Input: dimensioned drawing with shaded views. Units: mm. Origin: part minimum x, y, z. Give positions to 0.01 mm unless a question says otherwise; leave off trailing zeros. Order: outer loops, then holes, each group sorted by start corner. A loop starts at its lowest first (then second) coordinate and runs counter-clockwise, first axis right, second up.
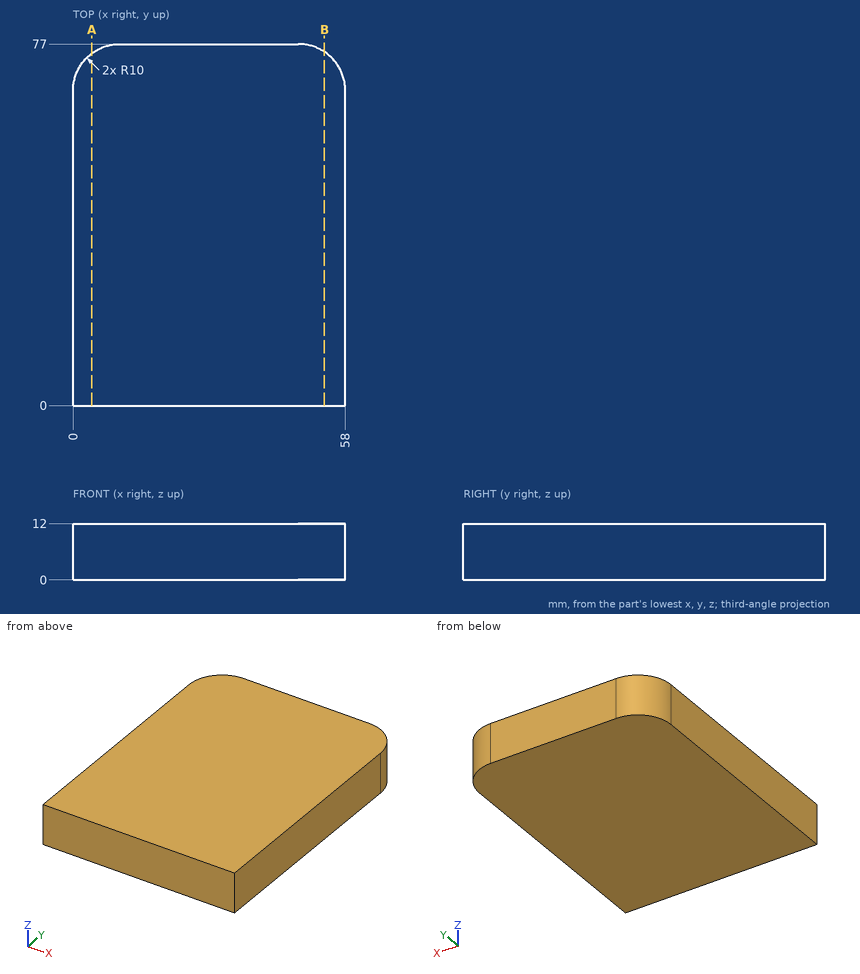
1) Line query: probe 1 along Y at (x, z) = (9.5, 0.75); probe 2 along Y at (x, z) = (49, 1.75); probe 3 along X at (y, z) = (71, 3.5). Output: solid intervals per line, ascending.
2) Cut plane A-A (x = 4). Return the cut outline in (y, z).
3) Cut plane B-B (x = 53.5). Return the cut outline in (y, z), then the cut area to 3 significant figures.
Geometry says:
1. probe 1: y = 0 to 76.99
1. probe 2: y = 0 to 76.95
1. probe 3: x = 0.83 to 57.17
2. outline: (0, 0) - (75, 0) - (75, 12) - (0, 12) - close
3. outline: (0, 0) - (75.35, 0) - (75.35, 12) - (0, 12) - close
3. area: 904 mm2
